from build123d import *

# Parameters (mm, degrees)
BOSS_EXTRUDE1_DEPTH = 100
SKETCH3_W           = 38
SKETCH3_H           = 122.430323754
CUT_EXTRUDE1_DEPTH  = 18
SKETCH4_R           = 13
CUT_EXTRUDE2_DEPTH  = 60


with BuildPart() as part:
    # Sketch2 → Boss-Extrude1 (new, symmetric)
    with BuildSketch(Plane.XY):
        Polygon((0, 0), (0, 74.558809371), (40, 74.558809371), (40, 14.558809371), align=None)
    extrude(amount=BOSS_EXTRUDE1_DEPTH, both=True)

    # Sketch3 → Cut-Extrude1 (cut)
    with BuildSketch(Plane.ZY):
        with Locations((-65, 44.558809371)):
            Rectangle(SKETCH3_W, SKETCH3_H)
    cut_extrude1 = extrude(amount=-CUT_EXTRUDE1_DEPTH, mode=Mode.SUBTRACT)

    # Mirror1: Cut-Extrude1 across plane
    add(cut_extrude1.mirror(Plane.XY), mode=Mode.SUBTRACT)

    # Sketch4 → Cut-Extrude2 (cut)
    with BuildSketch(Plane(origin=(0, 0, 0), x_dir=(0, 0, -1), z_dir=(1, 0, 0))):
        with Locations(Location((65, 44.558809371, 0), (0, 0, 180))):
            Circle(SKETCH4_R)
        with Locations(Location((-65, 44.558809371, 0), (0, 0, 180))):
            Circle(SKETCH4_R)
    extrude(amount=CUT_EXTRUDE2_DEPTH, mode=Mode.SUBTRACT)


solid = part.part
The listing builds one solid part. Answer for the finished solid, in the listing's coordinates (mm). A direction names the side the tool comes from. Coordinates: 2 decimals unless noted, no trailing zeros. Write each loop counter-clockwise with the first axis right and the second up, starting at its lowest first coordinate (ties: lowest second). Pieces come first, ordered by that corner, then holes. Notation, with made-up numbers: M 31,-39 L 89,-39 A28 ccw 89,-18 Z; hole C 72.5,8.5 d2. An arc over 180 degrees is marked long. Put each result on its own line as item: value. Start each with the question number.
1. A cutting plane is placed at C-C on x = 28. Write down the section's boundary in (y, z), then the cut area to 3 significant figures.
2. A cutting plane is placed at D-D on y = 29.5. Write down the section's boundary in (x, z), then the cut area to 3 significant figures.
3. Consider line 1 (Z direction, x = 6.5, y = 6.5); line 2 (Z direction, x = 24, y = 50); line 3 (X direction, y = 28, z = -58.5). Determine where each line is inside the solid, lowest interval first. Write a range as from..to.
4. Flat-ended cylindrical pins translate along their axes: P1, Ø10, axis at x = 7, z = 9, coming from the -Y side; P2, Ø11.5, axis at y = 32.5, z = -59.5, coming from the -X side. Find the tip coordinate at first contact, or state that the pin passes through.
5. For a pull along Y with two mould halves and no side action, classify faces 1 (the cylindrical face through (28.85, 57.25, 62.18)), 2 (the flat face through (20.28, 7.38, 1.4)), 3 (the cylindrical face through (28.846, 52.469, -75.316)), 4 (the flat face through (18, 33, -74)) as pulls with the +Y half, pulls with the -Y half, needs draft (parallel to the pull), parting line crosses it, or undercut.
6. A cutting plane is placed at A-A on z = -65. Write down the section's boundary in (x, y), then the cut area to 3 significant figures.
7. Which of the six approach directions +Z, -Z, +X, -X, +Y, -Y give full straight-line access (tool end or side, diameter ignored) to faces 5 (the flat face through (18, 33, 74)), 6 (the flat face through (20, 38, 100))?
8. A cutting plane is placed at B-B on y = 53. Write down the section's boundary in (x, z).
Resolved:
1. outline: M 10.19,-100 L 74.56,-100 L 74.56,100 L 10.19,100 Z; hole C 44.56,-65 d26; hole C 44.56,65 d26
1. area: 11,800 mm2
2. outline: M 0,-100 L 40,-100 L 40,100 L 0,100 L 0,84 L 18,84 L 18,46 L 0,46 L 0,-46 L 18,-46 L 18,-84 L 0,-84 Z
2. area: 6,630 mm2
3. line 1: z = -100..-84, -46..46, 84..100
3. line 2: z = -100..-76.81, -53.19..53.19, 76.81..100
3. line 3: x = 18..40
4. P1: stops at y = 0.73
4. P2: stops at x = 18
5. face 1: undercut
5. face 2: pulls with the -Y half
5. face 3: undercut
5. face 4: needs draft
6. outline: M 18,6.55 L 40,14.56 L 40,31.56 L 18,31.56 Z; M 18,57.56 L 40,57.56 L 40,74.56 L 18,74.56 Z
6. area: 836 mm2
7. face 5: -X, +Y, -Y
7. face 6: +Z, +X, -X, +Y, -Y
8. outline: M 0,-100 L 40,-100 L 40,-74.89 L 18,-74.89 L 18,-84 L 0,-84 Z; M 0,-46 L 18,-46 L 18,-55.11 L 40,-55.11 L 40,55.11 L 18,55.11 L 18,46 L 0,46 Z; M 0,84 L 18,84 L 18,74.89 L 40,74.89 L 40,100 L 0,100 Z
